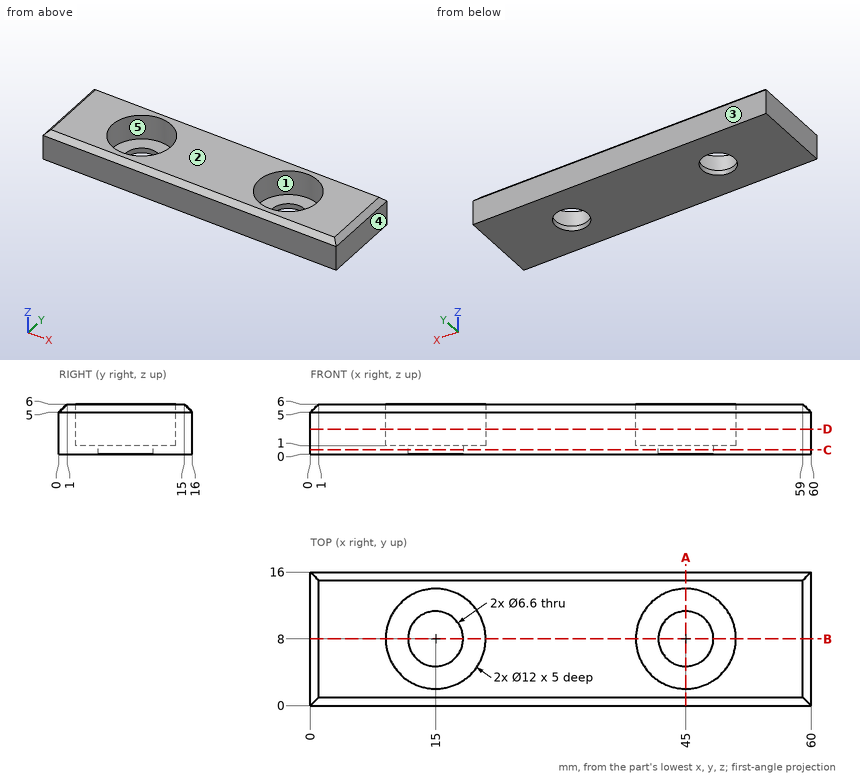
Print and shaded views of the part. All mm, measured from the part's lowest x, y and z. A direction names the side the tool comes from. Round coordinates to 2 decimals unless told otherwise and drop trailing zeros. Write each loop counter-clockwise with the first axis right and the second up, starting at its lowest first coordinate (ties: lowest second). Pieces come first, ordered by that corner, then holes. Notation, with made-up numbers: (-40, 15) - (-16, 15) arc R29 ccw to (-16, 53) - close; hole circle Ø5 at (-13, 0). An arc over 180 degrees is marked (long way). One line per question, with ' | ' between items.
1. Band-saw the part on D-D, the plane z = 3. Write the cut outline in (x, y).
Results are:
outline: (0, 0) - (60, 0) - (60, 16) - (0, 16) - close; hole circle Ø12 at (15, 8); hole circle Ø12 at (45, 8)
2. Drill centre lines: line 1 along Y through (x, z) = (45, 3.6); line 2 along X through (y, z) = (10.5, 3.5); line 3 along Y through (x, z) = (45, 0.75). Where is each one in solid material? Low to high. Write a range as from..to.
Results are:
line 1: 0..2, 14..16 | line 2: 0..9.55, 20.45..39.55, 50.45..60 | line 3: 0..4.7, 11.3..16
3. Band-saw the part on A-A, the plane x = 45. Write the cut outline in (y, z), and give its area (3 significant figures).
Results are:
outline: (0, 0) - (4.7, 0) - (4.7, 1) - (2, 1) - (2, 6) - (1, 6) - (0, 5) - close; (11.3, 0) - (16, 0) - (16, 5) - (15, 6) - (14, 6) - (14, 1) - (11.3, 1) - close | area: 28.4 mm^2
4. Band-saw the part on B-B, the plane y = 8. Write the cut outline in (x, z), and give its area (3 significant figures).
Results are:
outline: (0, 0) - (11.7, 0) - (11.7, 1) - (9, 1) - (9, 6) - (1, 6) - (0, 5) - close; (18.3, 0) - (41.7, 0) - (41.7, 1) - (39, 1) - (39, 6) - (21, 6) - (21, 1) - (18.3, 1) - close; (48.3, 0) - (60, 0) - (60, 5) - (59, 6) - (51, 6) - (51, 1) - (48.3, 1) - close | area: 226 mm^2
5. Tool access for the marked faces 1 and 2: list every direction of +Z, -Z, +X, -X, +Y, -Y with a clear straight run to the whole face (end or side of a thin tool).
Results are:
face 1: +Z | face 2: +Z, +X, -X, +Y, -Y
6. Band-saw the part on C-C, the plane z = 0.5. Write the cut outline in (x, y), and give its area (3 significant figures).
Results are:
outline: (0, 0) - (60, 0) - (60, 16) - (0, 16) - close; hole circle Ø6.6 at (15, 8); hole circle Ø6.6 at (45, 8) | area: 892 mm^2
7. Mould opens along Y. For the marked faces 3, 4 and 5 say: released by +Y, released by -Y, zero draft, split by the parting line, or undercut.
Results are:
face 3: released by +Y | face 4: zero draft | face 5: undercut
